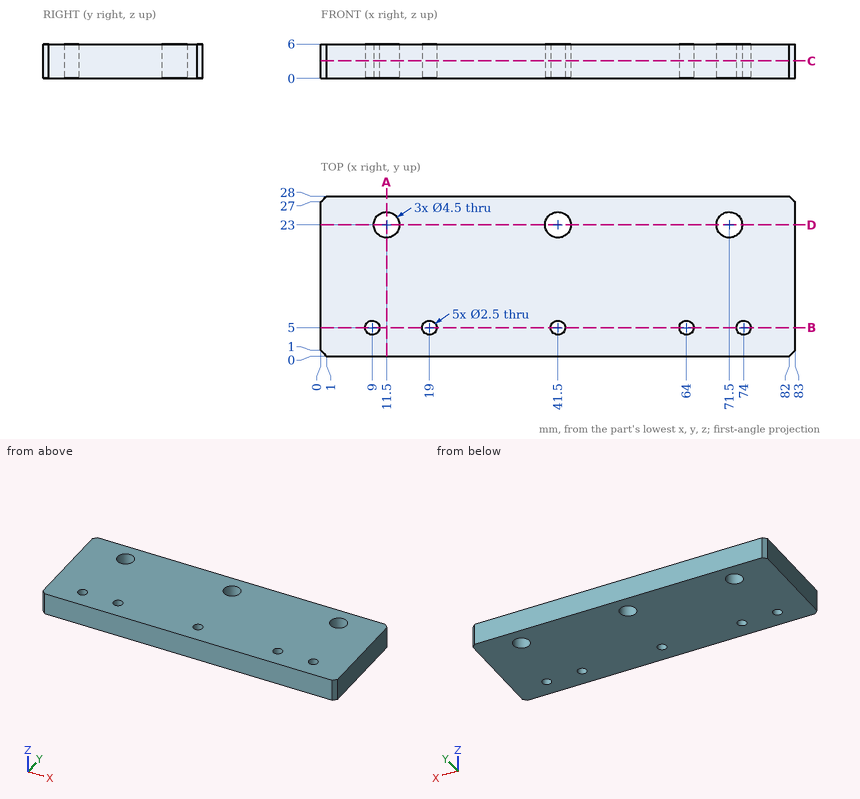
Design review of the part shown in the three views and the two pictorial views. Dimensions are in mm from the part's minimum x, y and z. Coordinates: 2 decimals unless noted, no trailing zeros. Write each loop counter-clockwise with the first axis right and the second up, starting at its lowest first coordinate (ties: lowest second). Pieces come first, ordered by that corner, then holes.
1) We need section D-D on y = 23. State the section outline as (x, z) points, then the cut area to 3 significant figures.
2) We need section C-C on z = 3.05. Count the separate pieces of the cut face and the enclosed holes in it, then the cut area to 3 significant figures.
3) Clearance check with a flat-ended pin moving along its axis: pin 1 Ø4 at (x, y) = (74, 5) entering from +Z. State where the tip first meets the part, or that it passes through.
4) We need section B-B on y = 5. State the section outline as (x, z) points.
5) To check wall thickness, follow probe 1 along Y at (x, z) = (11.5, 3.4); probe 2 along Y at (x, z) = (41.5, 2.5); probe 3 along Y at (x, z) = (64, 4.2). State the ranges of each line that lie inside material, in increasing order.
6) We need section A-A on x = 11.5. State the section outline as (y, z) points, then the cut area to 3 significant figures.
Answer list:
1. outline: (0, 0) - (9.25, 0) - (9.25, 6) - (0, 6) - close; (13.75, 0) - (39.25, 0) - (39.25, 6) - (13.75, 6) - close; (43.75, 0) - (69.25, 0) - (69.25, 6) - (43.75, 6) - close; (73.75, 0) - (83, 0) - (83, 6) - (73.75, 6) - close
1. area: 417 mm2
2. separate pieces: 1
2. enclosed holes: 8
2. area: 2,250 mm2
3. pin 1: stops at z = 6
4. outline: (0, 0) - (7.75, 0) - (7.75, 6) - (0, 6) - close; (10.25, 0) - (17.75, 0) - (17.75, 6) - (10.25, 6) - close; (20.25, 0) - (40.25, 0) - (40.25, 6) - (20.25, 6) - close; (42.75, 0) - (62.75, 0) - (62.75, 6) - (42.75, 6) - close; (65.25, 0) - (72.75, 0) - (72.75, 6) - (65.25, 6) - close; (75.25, 0) - (83, 0) - (83, 6) - (75.25, 6) - close
5. probe 1: y = 0 to 20.75, 25.25 to 28
5. probe 2: y = 0 to 3.75, 6.25 to 20.75, 25.25 to 28
5. probe 3: y = 0 to 3.75, 6.25 to 28
6. outline: (0, 0) - (20.75, 0) - (20.75, 6) - (0, 6) - close; (25.25, 0) - (28, 0) - (28, 6) - (25.25, 6) - close
6. area: 141 mm2
